Print and shaded views of the part. All mm, measured from the part's lowest x, y and z. A direction names the side the tool comes from. Round coordinates to 2 decimals unless told otherwise and drop trailing zeros. Write each loop counter-clockwise with the first axis right and the second up, starting at its lowest first coordinate (ties: lowest second). Pieces come first, ordered by that corner, then holes. Notation, with made-up numbers: (-24, 78) -> (27, 78) arc R37 cw to (27, 114) -> close; hole circle Ø5 at (-26, 57.25). An arc over 180 degrees is marked (long way). Use CSV: the item, a comma, the result in double quotes. Start each with the question number.
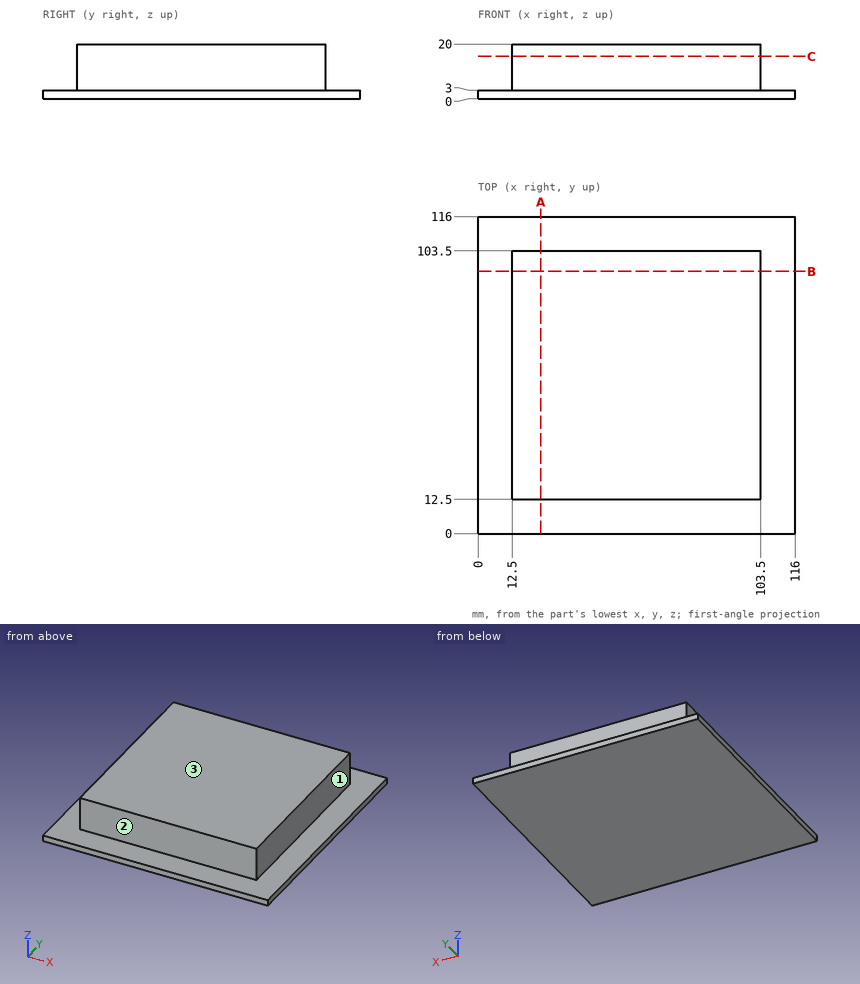
1. Flat gauge pins, fed straight in: pin 1 (2 mm diameter, centred on y = 79.5, z = 17, fed in from -X); pin 2 (5 mm diameter, centred on x = 65, z = 9, fed in from +Y); pin 3 (2 mm diameter, centred on x = 68.5, z = 16, fed in from -Y). Where does each tip first touch, or does it go through?
2. Band-saw the part on A-A (x = 23). List the corners of the cut face in (y, z), then the cut area to 4 significant figures.
3. Drill centre lines: line 1 along Z through (x, y) = (107, 72); line 2 along X through (y, z) = (73, 8.5). Where is each one in solid material? Low to high. Write a range as [from, to].
4. Which spindle directions (+Z, -Z, +X, -X, +Y, -Y) get a long thin tool onto all of the face, cutting with end or side? Do the marked faces 1, 2 and 3. Say none if no direction does.
5. Band-saw the part on C-C (z = 15.5). List the corners of the cut face in (x, y).
Answers below:
1,pin 1,"stops at x = 12.5"
1,pin 2,"stops at y = 103.5"
1,pin 3,"stops at y = 12.5"
2,outline,"(0, 0) -> (116, 0) -> (116, 3) -> (103.5, 3) -> (103.5, 20) -> (12.5, 20) -> (12.5, 3) -> (0, 3) -> close"
2,area,"1,895 mm^2"
3,line 1,"z = [0, 3]"
3,line 2,"x = [12.5, 103.5]"
4,face 1,"+Z, +X, +Y, -Y"
4,face 2,"+Z, +X, -X, -Y"
4,face 3,"+Z, +X, -X, +Y, -Y"
5,outline,"(12.5, 12.5) -> (103.5, 12.5) -> (103.5, 103.5) -> (12.5, 103.5) -> close"
